from build123d import *

# Parameters (mm, degrees)
BOSS_EXTRUDE3_DEPTH = 5
SKETCH3_R           = 1
CUT_EXTRUDE1_DEPTH  = 10


with BuildPart() as part:
    # Sketch1 → Boss-Extrude3 (new body)
    with BuildSketch(Plane.XY):
        with BuildLine():
            Line((26.130187968, 101.696672889), (28.618777298, 111.382070307))
            Line((28.618777298, 111.382070307), (31.107366629, 121.067467725))
            Line((31.107366629, 121.067467725), (33.595955959, 130.752865143))
            ThreePointArc((33.595955959, 130.752865143), (27.860620179, 132.093852405), (22.072250126, 133.183391511))
            ThreePointArc((22.072250126, 133.183391511), (19.849400241, 133.53277242), (17.62103595, 133.845056285))
            Line((17.62103595, 133.845056285), (16.315774028, 123.930607672))
            ThreePointArc((16.315774028, 123.930607672), (-7.533073444, 124.772804747), (-31.107366629, 121.067467725))
            Line((-31.107366629, 121.067467725), (-28.618777298, 111.382070307))
            ThreePointArc((-28.618777298, 111.382070307), (-5.016229547, 114.890545482), (18.802287144, 113.452518695))
            Line((18.802287144, 113.452518695), (17.167305653, 103.587082286))
            ThreePointArc((17.167305653, 103.587082286), (21.669371251, 102.739662982), (26.130187968, 101.696672889))
        make_face()
    extrude(amount=BOSS_EXTRUDE3_DEPTH)

    # Sketch3 → Cut-Extrude1 (cut)
    with BuildSketch(Plane(origin=(0, 0, 0), x_dir=(-1, 0, 0), z_dir=(0, 0, -1))):
        with Locations((25.988912996, 117.220204748)):
            Circle(SKETCH3_R)
    extrude(amount=-CUT_EXTRUDE1_DEPTH, mode=Mode.SUBTRACT)


solid = part.part
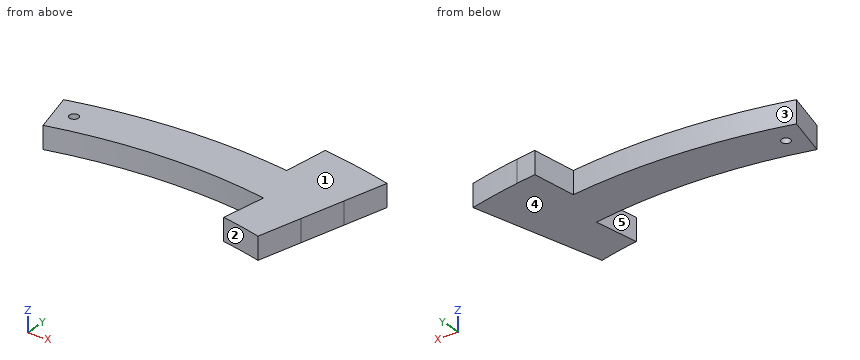
Read the model definition and answer for the solid it produces. Units are mm, in the model's axes. Face numbers are marked on the shaded views. A direction names the side the tool comes from. Coordinates: 2 decimals unless noted, no trailing zeros. Loops run counter-clockwise (first coordinate to the right, second up) from the corner with the lowest first, then second, coordinate; pieces in that order, holes last. Notation, with made-up numbers: (-36.5, -17) - (-29.5, -17) arc R36 ccw to (-29.5, 19) - close; hole circle Ø6 at (17, -2). An arc over 180 degrees is marked (long way). Answer in a Markdown table with one row per item.
Q1. Find section B-B on x = -6. Write down the section's boundary in (y, z), plus the area to 3 significant figures.
Here are the results:
| item | result |
|---|---|
| outline | (114.84, 0) - (124.86, 0) - (124.86, 5) - (114.84, 5) - close |
| area | 50.1 mm^2 |
Q2. Find section C-C on y = 126.5. Write down the section's boundary in (x, z).
Here are the results:
| item | result |
|---|---|
| outline | (16.65, 0) - (32.5, 0) - (32.5, 5) - (16.65, 5) - close |
Q3. Given P1, Ø1.5, axis at y = 106.5, z = 3, coming from the -X side, flat-ended and moving along its own axis, determine where the tip first touches the part or whether it passes through.
Here are the results:
| item | result |
|---|---|
| P1 | stops at x = 17.53 |
Q4. Straight lines are drawn through the part: line 1 along X through (y, z) = (117.5, 0.8); line 2 along X through (y, z) = (115.5, 3.1); line 3 along Y through (x, z) = (-24, 2.75). For each, find the intervals that lie inside material, in ascending order. Write a range as [from, to].
Here are the results:
| item | result |
|---|---|
| line 1 | x = [-30.19, -26.95], [-25.03, 30.19] |
| line 2 | x = [-29.68, 29.68] |
| line 3 | y = [112.47, 122.67] |
Q5. The mould has two halves that part along X. Classify the marked faces 1, 2 and 3: pulls with the +X half, pulls with the -X half, needs draft (parallel to the pull), parting line crosses it, or undercut.
Here are the results:
| item | result |
|---|---|
| face 1 | needs draft |
| face 2 | pulls with the -X half |
| face 3 | undercut |
Q6. Find section A-A on z = 1. Write down the section's boundary in (x, y).
Here are the results:
| item | result |
|---|---|
| outline | (-31.11, 121.07) - (-28.62, 111.38) arc R115 cw to (18.8, 113.45) - (17.17, 103.59) arc R105 cw to (26.13, 101.7) - (33.6, 130.75) arc R135 ccw to (22.07, 133.18) arc R135 ccw to (17.62, 133.85) - (16.32, 123.93) arc R125 ccw to start; hole circle Ø2 at (-25.99, 117.22) |
Q7. For the marked faces 4 and 5, determine the directions among +Z, -Z, +X, -X, +Y, -Y from which every point of the face is accessible in a straight line to the end or side of a thin tool.
Here are the results:
| item | result |
|---|---|
| face 4 | -Z, +X, -X, +Y, -Y |
| face 5 | +Z, -Z |
